from build123d import *

# Parameters (mm, degrees)
BOSS_EXTRUDE1_DEPTH = 24
SKETCH2_W           = 5
SKETCH2_H           = 8
CUT_EXTRUDE1_DEPTH  = 64
SKETCH3_R           = 3
CUT_EXTRUDE2_DEPTH  = 35
SKETCH4_R           = 14.1
CUT_EXTRUDE3_DEPTH  = 35
CHAMFER1_SIZE       = 1
CHAMFER2_SIZE       = 3


with BuildPart() as part:
    # Sketch1 → Boss-Extrude1 (new body)
    with BuildSketch(Plane(origin=(0, 0, 0), x_dir=(1, 0, 0), z_dir=(0, 1, 0))):
        with BuildLine():
            Line((-24, 19), (-24, 8))
            ThreePointArc((-24, 8), (-21.656854249, 2.343145751), (-16, 0))
            Line((-16, 0), (16, 0))
            ThreePointArc((16, 0), (21.656854249, 2.343145751), (24, 8))
            Line((24, 8), (24, 19))
            Line((24, 19), (32, 19))
            Line((32, 19), (32, 34))
            Line((32, 34), (26.5, 34))
            Line((26.5, 34), (26.5, 44))
            Line((26.5, 44), (-26.5, 44))
            Line((-26.5, 44), (-26.5, 34))
            Line((-26.5, 34), (-32, 34))
            Line((-32, 34), (-32, 19))
            Line((-32, 19), (-24, 19))
        make_face()
    extrude(amount=BOSS_EXTRUDE1_DEPTH)

    # Sketch2 → Cut-Extrude1 (cut)
    with BuildSketch(Plane.ZY.offset(26.5)):
        with Locations((-41.5, 12)):
            Rectangle(SKETCH2_W, SKETCH2_H)
    extrude(amount=-CUT_EXTRUDE1_DEPTH, mode=Mode.SUBTRACT)

    # Sketch3 → Cut-Extrude2 (cut)
    with BuildSketch(Plane(origin=(0, 0, -39), x_dir=(-1, 0, 0), z_dir=(0, 0, -1))):
        with Locations((-12, 12)):
            Circle(SKETCH3_R)
        with Locations(Location((12, 12, 0), (0, 0, 180))):
            Circle(SKETCH3_R)
    extrude(amount=-CUT_EXTRUDE2_DEPTH, mode=Mode.SUBTRACT)

    # Sketch4 → Cut-Extrude3 (cut)
    with BuildSketch(Plane.XZ):
        with Locations(Location((0, -26.5, 0), (0, 0, 270))):
            Circle(SKETCH4_R)
    extrude(amount=-CUT_EXTRUDE3_DEPTH, mode=Mode.SUBTRACT)

    # Chamfer1
    chamfer1_edges = [part.edges().sort_by_distance(p)[0] for p in [
        (-26.5, 20, -44),
        (26.5, 20, -44),
        (-26.5, 4, -44),
        (26.5, 4, -44),
        (0, 8, -44),
        (0, 16, -44),
    ]]
    chamfer(chamfer1_edges, length=CHAMFER1_SIZE)

    # Chamfer2
    chamfer2_edges = [part.edges().sort_by_distance(p)[0] for p in [
        (0, 0, -12.4),
    ]]
    chamfer(chamfer2_edges, length=CHAMFER2_SIZE)


solid = part.part
Geometry check sheet. Reference: the model listing, model coordinates, mm. A direction names the side the tool comes from. Give positions to 0.01 mm unless a question says otherwise; leave off trailing zeros. Order: outer loops, then holes, each group sorted by start corner. A loop starts at its lowest first (then second) coordinate and runs counter-clockwise, first axis right, second up.
1. Scan lines: line 1 (X direction, y = 8.25, z = -26); line 2 (X direction, y = 10.75, z = -9.5); line 3 (Y direction, x = 12, z = -14). Record each from-to range of solid material in increasing order.
Completed:
line 1: x = -32 to -14.09, 14.09 to 32
line 2: x = -24 to -14.73, -9.27 to 9.27, 14.73 to 24
line 3: y = 0 to 9, 15 to 24
2. Depth check by flat-ended pin: pin 1 (2.5 mm diameter, centred on x = -20.5, y = 12, fed in from -Z); pin 2 (3.5 mm diameter, centred on y = 15, z = -14.5, fed in from +X); pin 3 (4.5 mm diameter, centred on y = 17, z = -39.5, fed in from -X). Enter the tip coordinate at first touch or a pass-through.
Completed:
pin 1: stops at z = -39
pin 2: stops at x = 24
pin 3: stops at x = -26.5
3. Sectioned sample at C-C (z = -26.5). Record the boundary of the cut face in (x, y).
Completed:
outline: (-32, 0) - (-17.1, 0) - (-14.1, 3) - (-14.1, 9.86) arc R3 cw to (-14.1, 14.14) - (-14.1, 24) - (-32, 24) - close; (14.1, 3) - (17.1, 0) - (32, 0) - (32, 24) - (14.1, 24) - (14.1, 14.14) arc R3 cw to (14.1, 9.86) - close
4. Access from +Z, -Z, +X, -X, +Y, -Y to the whole of each face (thin tool, end or side, straight path). Record for faces 4 (the face through (12, 12, -4)), 5 (the face through (29, 12, -34)), 6 (the face through (24, 12, -13)), 7 (the face through (19, 12, -39)), 8 (the face through (-29, 12, -34)).
Completed:
face 4: -Z
face 5: -Z, +X, +Y, -Y
face 6: +Z, +X, +Y, -Y
face 7: -Z, +X, -X
face 8: -Z, -X, +Y, -Y
5. Draft check along Y on faces 1 (the face through (0.626, 2.854, -12.268)), 2 (the face through (-19, 12, -39)), 3 (the face through (26.5, 12, -38)). Enter one of: pulls with the +Y half, pulls with the -Y half, needs draft (parallel to the pull), parting line crosses it, or undercut.
Completed:
face 1: pulls with the -Y half
face 2: undercut
face 3: needs draft
6. Sectioned sample at A-A (x = 0). Record the boundary of the cut face in (y, z).
Completed:
outline: (0, -44) - (7, -44) - (8, -43) - (8, -40.6) - (3, -40.6) - (0, -43.6) - close; (0, -9.4) - (3, -12.4) - (24, -12.4) - (24, 0) - (0, 0) - close; (16, -43) - (17, -44) - (24, -44) - (24, -40.6) - (16, -40.6) - close
7. Sectioned sample at D-D (y = 12). Record the boundary of the cut face in (x, z).
Completed:
outline: (-32, -34) - (-26.5, -34) - (-26.5, -39) - (-15, -39) - (-15, -4) - (-9, -4) - (-9, -15.65) arc R14.1 cw to (9, -15.65) - (9, -4) - (15, -4) - (15, -39) - (26.5, -39) - (26.5, -34) - (32, -34) - (32, -19) - (24, -19) - (24, -8) arc R8 ccw to (16, 0) - (-16, 0) arc R8 ccw to (-24, -8) - (-24, -19) - (-32, -19) - close; (-9, -39) - (-6.52, -39) arc R14.1 cw to (-9, -37.35) - close; (6.52, -39) - (9, -39) - (9, -37.35) arc R14.1 cw to start
8. Sectioned sample at B-B (y = 20.5). Record the boundary of the cut face in (x, z).
Completed:
outline: (-32, -34) - (-26.5, -34) - (-26.5, -43) - (-25.5, -44) - (25.5, -44) - (26.5, -43) - (26.5, -34) - (32, -34) - (32, -19) - (24, -19) - (24, -8) arc R8 ccw to (16, 0) - (-16, 0) arc R8 ccw to (-24, -8) - (-24, -19) - (-32, -19) - close; hole circle Ø28.2 at (0, -26.5)
